Input: part model. Units: mm. Frame: model coordinates. A direction names the side the tool comes from. Round coordinates to 2 decimals unless told otherwise and drop trailing zeros. Loops run counter-clockwise (first coordinate to the right, second up) from the corner with the lowest first, then second, coordinate; pieces in that order, holes last. Notation, with made-up numbers: (89.5, -18) -> (97.5, -18) arc R28 cw to (97.5, 10) -> close; hole circle Ø7 at (81, -26). An arc over 180 degrees is marked (long way). Answer in a Markdown table with one row per item. Add a question column.
Q1. Section D-D, the plane y = 17.5. Output: boundary loops of the cut face in (x, z).
Q2. Section B-B, the plane y = 36. Output: boundary loops of the cut face in (x, z).
Q3. Section A-A, the plane z = 0. Output: boundary loops of the cut face in (x, y).
Q4. Section C-C, the plane x = 0. Output: boundary loops of the cut face in (y, z).
Q5. Pin query (flat end, axial travel): pin 1 (5 mm diameter, centred on y = 9, z = -3.5, fed in from -X); pin 2 (8.5 mm diameter, centred on x = 6.5, y = 38.5, fed in from -Z); pin 3 (7 mm diameter, centred on y = 46, z = -22, fed in from -X); pin 4 (1 mm diameter, centred on x = -25.5, y = 22, fed in from +Z). Return the tip coordinate at first contact, or that it passes through.
Q6. Reachability of faces 1 (the face through (9, 42, 12)), 2 (the face through (11.5, 10, 0)), 3 (the face through (-14, 42, 21)), 4 (the face through (14, 43, -21)), 5 (the face through (-22, 18, 0)) from +Z, -Z, +X, -X, +Y, -Y: full face, straight path, thin tool, end or side. Return the list, or none.
Q7. Mould query, pull axis X, two halves, no side actions, for faces 6 (the face through (-22, 35, 16)), 7 (the face through (22, 35, 16)), 8 (the face through (0, 19, 25)), 9 (the face through (-14, 42, -21)). Classes: pulls with the +X half, pulls with the -X half, needs draft (parallel to the pull), parting line crosses it, or undercut.
Q8. Ray query, L1, parallel to Z at x = 16, y = 15.5; L2, parallel to X at y = 44.5, z = 14; L3, parallel to Z at x = -9.5, y = 47. Return the intervals inside material, ascending. Write a range as from..to.
```python
from build123d import *

# Parameters (mm, degrees)
BASE_BLOCK_DEPTH         = 20
UPRIGHTS_DEPTH           = 18
UPRIGHT_NOTCH_DEPTH      = 9
UNDERSIDE_SLOT_PROFILE_W = 30
UNDERSIDE_SLOT_PROFILE_H = 10
UNDERSIDE_SLOT_DEPTH     = 82.737384348
SADDLE_CUT_PROFILE_W     = 23
SADDLE_CUT_PROFILE_H     = 14
SADDLE_CUT_DEPTH         = 57.621550668
UPRIGHT_SLOT_PROFILE_W   = 44
UPRIGHT_SLOT_PROFILE_H   = 14
UPRIGHT_SLOT_CUT_DEPTH   = 5


with BuildPart() as part:
    # Base Block Profile → Base Block (new body)
    with BuildSketch(Plane(origin=(0, 0, 0), x_dir=(1, 0, 0), z_dir=(0, 1, 0))):
        with BuildLine():
            Line((-25, 25), (25, 25))
            Line((25, 25), (41, 18))
            Line((41, 18), (41, 13))
            ThreePointArc((41, 13), (28, 0), (41, -13))
            Line((41, -13), (41, -18))
            Line((41, -18), (25, -25))
            Line((25, -25), (-25, -25))
            Line((-25, -25), (-41, -18))
            Line((-41, -18), (-41, -13))
            ThreePointArc((-41, -13), (-28, 0), (-41, 13))
            Line((-41, 13), (-41, 18))
            Line((-41, 18), (-25, 25))
        make_face()
    extrude(amount=BASE_BLOCK_DEPTH)

    # Uprights Profile → Uprights (add)
    with BuildSketch(Plane.XY.offset(25)):
        with BuildLine():
            Line((-22, 20), (-22, 50))
            Line((-22, 50), (-9, 50))
            Line((-9, 50), (-9, 35))
            ThreePointArc((-9, 35), (0, 26), (9, 35))
            Line((9, 35), (9, 50))
            Line((9, 50), (22, 50))
            Line((22, 50), (22, 20))
            Line((22, 20), (-22, 20))
        make_face()
    uprights = extrude(amount=-UPRIGHTS_DEPTH)

    # Upright Notch Profile → Upright Notch (cut)
    with BuildSketch(Plane.XY.offset(25)):
        with BuildLine():
            Line((-14, 50), (14, 50))
            Line((14, 50), (14, 35))
            ThreePointArc((14, 35), (0, 21), (-14, 35))
            Line((-14, 35), (-14, 50))
        make_face()
    upright_notch = extrude(amount=-UPRIGHT_NOTCH_DEPTH, mode=Mode.SUBTRACT)

    # Upright Notch Mirror: Uprights, Upright Notch across plane
    add(uprights.mirror(Plane.XY))
    add(upright_notch.mirror(Plane.XY), mode=Mode.SUBTRACT)

    # Underside Slot Profile → Underside Slot (cut, through all)
    with BuildSketch(Plane.XY.offset(25)):
        Rectangle(UNDERSIDE_SLOT_PROFILE_W, UNDERSIDE_SLOT_PROFILE_H)
    extrude(amount=-UNDERSIDE_SLOT_DEPTH, mode=Mode.SUBTRACT)

    # Saddle Cut Profile → Saddle Cut (cut, through all)
    with BuildSketch(Plane(origin=(0, 20, 0), x_dir=(1, 0, 0), z_dir=(0, 1, 0))):
        Rectangle(SADDLE_CUT_PROFILE_W, SADDLE_CUT_PROFILE_H)
    extrude(amount=-SADDLE_CUT_DEPTH, mode=Mode.SUBTRACT)

    # Upright Slot Profile → Upright Slot Cut (cut)
    with BuildSketch(Plane(origin=(0, 20, 0), x_dir=(1, 0, 0), z_dir=(0, 1, 0))):
        Rectangle(UPRIGHT_SLOT_PROFILE_W, UPRIGHT_SLOT_PROFILE_H)
    extrude(amount=-UPRIGHT_SLOT_CUT_DEPTH, mode=Mode.SUBTRACT)


solid = part.part
```
Answer block:
| question | item | result |
|---|---|---|
| 1 | outline | (-41, -18) -> (-25, -25) -> (25, -25) -> (41, -18) -> (41, -13) arc R13 cw to (41, 13) -> (41, 18) -> (25, 25) -> (-25, 25) -> (-41, 18) -> (-41, 13) arc R13 cw to (-41, -13) -> close; hole (-22, -7) -> (22, -7) -> (22, 7) -> (-22, 7) -> close |
| 2 | outline | (-22, -25) -> (-14, -25) -> (-14, -16) -> (-9, -16) -> (-9, -7) -> (-22, -7) -> close; (-22, 7) -> (-9, 7) -> (-9, 16) -> (-14, 16) -> (-14, 25) -> (-22, 25) -> close; (9, -16) -> (14, -16) -> (14, -25) -> (22, -25) -> (22, -7) -> (9, -7) -> close; (9, 7) -> (22, 7) -> (22, 25) -> (14, 25) -> (14, 16) -> (9, 16) -> close |
| 3 | outline | (-28, 0) -> (-15, 0) -> (-15, 5) -> (-11.5, 5) -> (-11.5, 15) -> (-22, 15) -> (-22, 20) -> (-28, 20) -> close; (11.5, 5) -> (15, 5) -> (15, 0) -> (28, 0) -> (28, 20) -> (22, 20) -> (22, 15) -> (11.5, 15) -> close |
| 4 | outline | (5, -25) -> (21, -25) -> (21, -16) -> (26, -16) -> (26, -7) -> (5, -7) -> close; (5, 7) -> (26, 7) -> (26, 16) -> (21, 16) -> (21, 25) -> (5, 25) -> close |
| 5 | pin 1 | x = -29.47 |
| 5 | pin 2 | z = -16 |
| 5 | pin 3 | x = -22 |
| 5 | pin 4 | through |
| 6 | face 1 | +Z, -Z, +Y |
| 6 | face 2 | +Y, -Y |
| 6 | face 3 | +Z, +Y |
| 6 | face 4 | -Z, +Y |
| 6 | face 5 | +Y |
| 7 | face 6 | pulls with the -X half |
| 7 | face 7 | pulls with the +X half |
| 7 | face 8 | needs draft |
| 7 | face 9 | undercut |
| 8 | L1 | -25..-7, 7..25 |
| 8 | L2 | -22..-9, 9..22 |
| 8 | L3 | -16..-7, 7..16 |
